from build123d import *

# Parameters (mm, degrees)
SKETCH1_W           = 300
SKETCH1_H           = 690
BOSS_EXTRUDE1_DEPTH = 700
SKETCH2_W           = 630
SKETCH2_H           = 150
CUT_EXTRUDE1_DEPTH  = 280
SKETCH3_W           = 630
SKETCH3_H           = 460
CUT_EXTRUDE2_DEPTH  = 280


with BuildPart() as part:
    # Sketch1 → Boss-Extrude1 (new body)
    with BuildSketch(Plane.XY):
        Rectangle(SKETCH1_W, SKETCH1_H)
    extrude(amount=BOSS_EXTRUDE1_DEPTH)

    # Sketch2 → Cut-Extrude1 (cut)
    with BuildSketch(Plane(origin=(150, 0, 0), x_dir=(0, 0, -1), z_dir=(1, 0, 0))):
        with Locations((-350, 250)):
            Rectangle(SKETCH2_W, SKETCH2_H)
    extrude(amount=-CUT_EXTRUDE1_DEPTH, mode=Mode.SUBTRACT)

    # Sketch3 → Cut-Extrude2 (cut)
    with BuildSketch(Plane(origin=(150, 0, 0), x_dir=(0, 0, -1), z_dir=(1, 0, 0))):
        with Locations((-350, -95)):
            Rectangle(SKETCH3_W, SKETCH3_H)
    extrude(amount=-CUT_EXTRUDE2_DEPTH, mode=Mode.SUBTRACT)


solid = part.part
Could you check a few things on this model? Use its own coordinates, in mm. A direction names the side the tool comes from. Coordinates: 2 decimals unless noted, no trailing zeros. Write each loop counter-clockwise with the first axis right and the second up, starting at its lowest first coordinate (ties: lowest second). Pieces come first, ordered by that corner, then holes. Notation, with made-up numbers: M 0.25,3.5 L 28.25,3.5 A27 ccw 28.25,20.5 Z; hole C 60.5,45.25 d6. An arc over 180 degrees is marked long. One line per question, with ' | ' between items.
1) I need wall thicknesses on probe 1 along Y at (x, z) = (-111, 483.5); probe 2 along Z at (x, y) = (-66, -26.5); probe 3 along X at (y, z) = (185, 368). Which ranges of each line are inside material? Lowest first, please. Write a range as [from, to].
Checks:
probe 1: [-345, -325], [135, 175], [325, 345] | probe 2: [0, 35], [665, 700] | probe 3: [-150, -130]
2) Imagine slicing it at C-C, the plane z = 202. Write out the boundary of the cut face in (x, y).
Checks:
outline: M -150,-345 L 150,-345 L 150,-325 L -130,-325 L -130,135 L 150,135 L 150,175 L -130,175 L -130,325 L 150,325 L 150,345 L -150,345 Z
3) Imagine slicing it at A-A, the plane x = -9.5. Write out the boundary of the cut face in (y, z).
Checks:
outline: M -345,0 L 345,0 L 345,700 L -345,700 Z; hole M -325,35 L 135,35 L 135,665 L -325,665 Z; hole M 175,35 L 325,35 L 325,665 L 175,665 Z
4) For faces 1 (the face through (-2, -345, 345)), 2 (the face through (-130, -92, 354)), which set-ups out of +Z, -Z, +X, -X, +Y, -Y let a thin tool reach every point of the face, with its end or its side?
Checks:
face 1: +Z, -Z, +X, -X, -Y | face 2: +X
5) For pin 1 Ø2 at (y, z) = (52, 149) entering from +X, with a flat end and sliding along its axis, tell me the tip position at first contact or that it passes through.
Checks:
pin 1: x = -130
6) If we mould it in two halves opening along Z, with no side actions, what happens to faces 3 (the face through (-2, 5, 0)), 4 (the face through (12, 135, 354)), 5 (the face through (12, -325, 354)), 6 (the face through (150, 152, 348))? For each: released by +Z, released by -Z, zero draft, split by the parting line, or undercut.
Checks:
face 3: released by -Z | face 4: undercut | face 5: undercut | face 6: zero draft
7) Imagine slicing it at B-B, the plane y = 68. Write out the boundary of the cut face in (x, z).
Checks:
outline: M -150,0 L 150,0 L 150,35 L -130,35 L -130,665 L 150,665 L 150,700 L -150,700 Z
